from build123d import *

# Parameters (mm, degrees)
BASE_PLATE_DEPTH    = 10
RIM_WALL_SKETCH_R   = 11.5
RIM_WALL_SKETCH_R_2 = 4.5
RIM_WALL_DEPTH      = 5
FORK_BLOCK_DEPTH    = 15


with BuildPart() as part:
    # Base Plate Profile Sketch → Base Plate (new body)
    with BuildSketch(Plane(origin=(0, 0, 0), x_dir=(1, 0, 0), z_dir=(0, 1, 0))):
        with BuildLine():
            ThreePointArc((-24.722478982, 82.179410314), (-27.300831577, 76.65011533), (-28.879861205, 70.757096532))
            Line((-28.879861205, 70.757096532), (-40.321517202, 5.868240888))
            ThreePointArc((-40.321517202, 5.868240888), (-39.227700653, 1.786061952), (-35.397478437, 0))
            Line((-35.397478437, 0), (32.684985637, 0))
            ThreePointArc((32.684985637, 0), (36.515207852, 1.786061952), (37.609024402, 5.868240888))
            Line((37.609024402, 5.868240888), (27.174016631, 65.048110745))
            ThreePointArc((27.174016631, 65.048110745), (27.174016631, 70.257556075), (28.95575187, 75.15283341))
            Line((28.95575187, 75.15283341), (23.980814684, 66.53598944))
            ThreePointArc((23.980814684, 66.53598944), (24.071961031, 65.528220723), (24.219593372, 64.527166212))
            Line((24.219593372, 64.527166212), (34.654601143, 5.347296355))
            ThreePointArc((34.654601143, 5.347296355), (34.217074523, 3.714424781), (32.684985637, 3))
            Line((32.684985637, 3), (-35.397478437, 3))
            ThreePointArc((-35.397478437, 3), (-36.929567324, 3.714424781), (-37.367093943, 5.347296355))
            Line((-37.367093943, 5.347296355), (-25.925437946, 70.236151999))
            ThreePointArc((-25.925437946, 70.236151999), (-24.481753715, 75.6240549), (-22.124402771, 80.679410314))
            Line((-22.124402771, 80.679410314), (-19.052558883, 86))
            Line((-19.052558883, 86), (-21.650635095, 87.5))
            Line((-21.650635095, 87.5), (-24.722478982, 82.179410314))
        make_face()
    extrude(amount=BASE_PLATE_DEPTH)

    # Rim Wall Sketch → Rim Wall (add)
    with BuildSketch(Plane(origin=(0, 0, 0), x_dir=(1, 0, 0), z_dir=(0, 1, 0))):
        with BuildLine():
            Line((21.650635095, 62.5), (-19.052558883, 86))
            Line((-19.052558883, 86), (-22.124402771, 80.679410314))
            ThreePointArc((-22.124402771, 80.679410314), (-24.481753715, 75.6240549), (-25.925437946, 70.236151999))
            Line((-25.925437946, 70.236151999), (-37.367093943, 5.347296355))
            ThreePointArc((-37.367093943, 5.347296355), (-36.929567324, 3.714424781), (-35.397478437, 3))
            Line((-35.397478437, 3), (32.684985637, 3))
            ThreePointArc((32.684985637, 3), (34.217074523, 3.714424781), (34.654601143, 5.347296355))
            Line((34.654601143, 5.347296355), (24.219593372, 64.527166212))
            ThreePointArc((24.219593372, 64.527166212), (24.071961031, 65.528220723), (23.980814684, 66.53598944))
            Line((23.980814684, 66.53598944), (21.650635095, 62.5))
        make_face()
        with Locations(Location((0, 20, 0), (0, 0, 270))):
            Circle(RIM_WALL_SKETCH_R, mode=Mode.SUBTRACT)
        with Locations(Location((0, 45, 0), (0, 0, 270))):
            Circle(RIM_WALL_SKETCH_R_2, mode=Mode.SUBTRACT)
    extrude(amount=RIM_WALL_DEPTH)

    # Fork Block Sketch → Fork Block (add)
    with BuildSketch(Plane(origin=(0, 0, 0), x_dir=(1, 0, 0), z_dir=(0, 1, 0))):
        Polygon((39.150635095, 92.810889132), (30.490381057, 97.810889132), (17.990381057, 76.160254038), (-7.990381057, 91.160254038), (4.509618943, 112.810889132), (-4.150635095, 117.810889132), (-21.650635095, 87.5), (21.650635095, 62.5), align=None)
    extrude(amount=FORK_BLOCK_DEPTH)


solid = part.part
For this review, take the finished solid that the model builds, in its own axes (mm). A direction names the side the tool comes from. Coordinates: 2 decimals unless noted, no trailing zeros. Order: outer loops, then holes, each group sorted by start corner. A loop starts at its lowest first (then second) coordinate and runs counter-clockwise, first axis right, second up. Notation, with made-up numbers: (16, 19.5) - (49, 19.5) arc R28 cw to (49, 52.5) - close; hole circle Ø11 at (15, 63). An arc over 180 degrees is marked (long way). Answer as CSV lines item,"result". Start each with the question number.
1) Add section A-A (y = 6.5). State the section outline as (x, z) points.
2) To check wall thickness, follow line 1 along Y through (x, z) = (2, -52); line 2 along X through (y, z) = (3.3, -20); line 3 along X through (y, z) = (12, -81). State the ranges of each line that lie inside material, in increasing order. Write a range as [from, to].
3) Draft analysis for pull direction X (two halves, no side actions). For faces 1 (the flat face through (4, 15, -84)), 2 (the flat face through (5.182, 7.395, -83.555)), 3 (the flat face through (32.465, 4.93, -35.044)), state which applies: +X half, -X half, draft (parallel to the pull), parting line (faces both ways), or undercut.
4) Add section B-B (z = -28.5). State the section outline as (x, y) points.
5) Machinability: for faces 4 (the flat face through (-1, 7, -3)), 5 (the flat face through (-1.83, 7.4, -101.83)), 6 (the cylindrical face through (-27.27, 4.93, -76.73)), 7 (the flat face through (8, 0, -47)), 8 (the flat face through (24.33, 7.4, -87.14)), which of the approach directions +Z, -Z, +X, -X, +Y, -Y give a long, thin tool a straight path to every point of the face, cutting with its end or side? Answer none if there is none.
6) Add section C-C (x = 0). State the section outline as (y, z) points.
7) Insertion check: P1, Ø5, axis at y = 4.5, z = -21.5, coming from the +X side; P2, Ø23.5, axis at x = -16, z = -29, coming from the +Y side; P3, Ø2.5, axis at x = -16, y = 6.5, coming from the -Z side. Each pin has a flat end and moves straight along its axis. Give the tip position at first contact, or say it passes through.
8) Add section D-D (x = -16). State the section outline as (y, z) points.
Result:
1,outline,"(-40.32, -5.87) - (-28.88, -70.76) arc R35 ccw to (-24.72, -82.18) - (-4.15, -117.81) - (4.51, -112.81) - (-7.99, -91.16) - (17.99, -76.16) - (30.49, -97.81) - (39.15, -92.81) - (28.96, -75.15) arc R15 cw to (27.17, -65.05) - (37.61, -5.87) arc R5 ccw to (32.68, 0) - (-35.4, 0) arc R5 ccw to start; hole (-37.37, -5.35) - (-25.93, -70.24) arc R32 ccw to (-22.12, -80.68) - (-19.05, -86) - (21.65, -62.5) - (23.98, -66.54) arc R18 cw to (24.22, -64.53) - (34.65, -5.35) arc R2 ccw to (32.68, -3) - (-35.4, -3) arc R2 ccw to start"
2,line 1,"[0, 5]"
2,line 2,"[-37.83, -11.5], [11.5, 35.12]"
2,line 3,"[-10.39, 9.61], [20.78, 32.33]"
3,face 1,"draft"
3,face 2,"undercut"
3,face 3,"+X half"
4,outline,"(-36.33, 0) - (-7.75, 0) - (-7.75, 5) - (-33.28, 5) - (-33.28, 10) - (-36.33, 10) - close; (7.75, 0) - (33.62, 0) - (33.62, 10) - (30.57, 10) - (30.57, 5) - (7.75, 5) - close"
5,face 4,"+Y"
5,face 5,"+Y, -Y"
5,face 6,"-Z, -X, +Y, -Y"
5,face 7,"+Z, -Z, +X, -X, -Y"
5,face 8,"-Z, +Y, -Y"
6,outline,"(0, -115.41) - (15, -115.41) - (15, -105) - (0, -105) - close; (0, -86.55) - (15, -86.55) - (15, -75) - (5, -75) - (5, -49.5) - (0, -49.5) - close; (0, -40.5) - (5, -40.5) - (5, -31.5) - (0, -31.5) - close; (0, -8.5) - (5, -8.5) - (5, -3) - (10, -3) - (10, 0) - (0, 0) - close"
7,P1,"x = 35.29"
7,P2,"y = 5"
7,P3,"z = -99.45"
8,outline,"(0, -97.29) - (15, -97.29) - (15, -84.24) - (5, -84.24) - (5, -3) - (10, -3) - (10, 0) - (0, 0) - close"
